The model under review builds one solid part; all positions refer to its coordinate system, in mm. Give positions to 0.01 mm unless a question says otherwise; leave off trailing zeros. Loops run counter-clockwise (first coordinate to the right, second up) from the corner with the lowest first, then second, coordinate; pieces in that order, holes last. Notation, with made-up numbers: (52, 49.5) -> (74, 49.5) arc R16 cw to (74, 57.5) -> close; hole circle Ø9 at (29.5, 70). An arc over 180 degrees is marked (long way). Write each question's results on one line, items separated by ' | '. Start each with the question number.
Q1. Mouldability with a two-part tool opening along Y and no side actions: class faces 1 (the face through (220, 0, 1)), 2 (the face through (3, 5, 2.5)), 3 (the face through (-205.23, 1.5, 1.23)) as released by +Y, released by -Y, zero draft, split by the parting line, or undercut.
Q2. We need section B-B (y = 0). Write out the cut boundary in (x, z).
Q3. We need section A-A (x = 0). Write out the cut boundary in (y, z).
Q4. Wall thickness on L1, parallel to X at y = 0.5, z = 0.2; L2, parallel to Y at x = 0, z = 1.95; L3, parallel to X at y = -4, z = 0.7: over which ranges is each line inside the solid? List them lowest first. Write a range as [from, to].
Q5. We need section C-C (z = 1.7). Write out the cut boundary in (x, y), plus the area to 3 significant figures.
Q6. Insertion check: pin 1 Ø6 at (x, y) = (-210, 0) entering from -Z. The pin has a flat end and moves straight along its axis. Give the tip position at first contact, or say it passes through.
from build123d import *

# Parameters (mm, degrees)
SKETCH1_R           = 5
BOSS_EXTRUDE1_DEPTH = 2.5


with BuildPart() as part:
    # Sketch1 → Boss-Extrude1 (new body)
    with BuildSketch(Plane.XY):
        with BuildLine():
            Line((-210, 10), (210, 10))
            ThreePointArc((210, 10), (220, 0), (210, -10))
            Line((210, -10), (-210, -10))
            ThreePointArc((-210, -10), (-220, 0), (-210, 10))
        make_face()
        with Locations((-210, 0)):
            Circle(SKETCH1_R, mode=Mode.SUBTRACT)
        with Locations((210, 0)):
            Circle(SKETCH1_R, mode=Mode.SUBTRACT)
        Circle(SKETCH1_R, mode=Mode.SUBTRACT)
    extrude(amount=BOSS_EXTRUDE1_DEPTH)


solid = part.part
Output:
1) face 1: split by the parting line | face 2: zero draft | face 3: undercut
2) outline: (-220, 0) -> (-215, 0) -> (-215, 2.5) -> (-220, 2.5) -> close; (-205, 0) -> (-5, 0) -> (-5, 2.5) -> (-205, 2.5) -> close; (5, 0) -> (205, 0) -> (205, 2.5) -> (5, 2.5) -> close; (215, 0) -> (220, 0) -> (220, 2.5) -> (215, 2.5) -> close
3) outline: (-10, 0) -> (-5, 0) -> (-5, 2.5) -> (-10, 2.5) -> close; (5, 0) -> (10, 0) -> (10, 2.5) -> (5, 2.5) -> close
4) L1: [-219.99, -214.97], [-205.03, -4.97], [4.97, 205.03], [214.97, 219.99] | L2: [-10, -5], [5, 10] | L3: [-219.17, -213], [-207, -3], [3, 207], [213, 219.17]
5) outline: (-210, -10) -> (210, -10) arc R10 ccw to (210, 10) -> (-210, 10) arc R10 ccw to start; hole circle Ø10 at (-210, 0); hole circle Ø10 at (0, 0); hole circle Ø10 at (210, 0) | area: 8,480 mm2
6) pin 1: through
